Design review of the part built by this model. Coordinates are the model's own, in mm. A direction names the side the tool comes from. Coordinates: 2 decimals unless noted, no trailing zeros. Loops run counter-clockwise (first coordinate to the right, second up) from the corner with the lowest first, then second, coordinate; pieces in that order, holes last. Notation, with made-up numbers: (-40, -20) -> (-21, -20) arc R34 cw to (-21, 12) -> close; hole circle Ø2 at (-30, 62). An arc over 180 degrees is marked (long way). Use CSV: the item, a comma, the result in double quotes.
```python
from build123d import *

# Parameters (mm, degrees)
SKETCH1_W                                = 34
SKETCH1_H                                = 45
BASE_EXTRUDE_DEPTH                       = 16
CUT_EXTRUDE1_DEPTH                       = 56.951622292
CBORE_FOR_M5_HEX_HEAD_SCREW1_D           = 6.6
CBORE_FOR_M5_HEX_HEAD_SCREW1_CBORE_D     = 12
CBORE_FOR_M5_HEX_HEAD_SCREW1_CBORE_DEPTH = 6
SKETCH3_R                                = 3
CUT_EXTRUDE4_DEPTH                       = 25
CHAMFER3_SIZE                            = 2
CHAMFER4_SIZE                            = 2
CBORE_FOR_M5_HEX_HEAD_SCREW2_D           = 6.6
CBORE_FOR_M5_HEX_HEAD_SCREW2_CBORE_D     = 12
CBORE_FOR_M5_HEX_HEAD_SCREW2_CBORE_DEPTH = 6
FILLET1_R                                = 1
FILLET2_R                                = 1
SKETCH13_W                               = 37.795873191
SKETCH13_H                               = 5.669380978
CUT_EXTRUDE5_DEPTH                       = 56.951622292


with BuildPart() as part:
    # Sketch1 → Base-Extrude (new body)
    with BuildSketch(Plane.XY):
        with Locations((0, 28.348638498)):
            Rectangle(SKETCH1_W, SKETCH1_H)
    extrude(amount=BASE_EXTRUDE_DEPTH)

    # Sketch2 → Cut-Extrude1 (cut, through all)
    with BuildSketch(Plane.XY.offset(16)):
        Polygon((-4, 38.848638498), (4, 38.848638498), (4, 42.848638498), (12, 50.848638498), (-12, 50.848638498), (-4, 42.848638498), align=None)
    extrude(amount=-CUT_EXTRUDE1_DEPTH, mode=Mode.SUBTRACT)

    # CBORE for M5 Hex Head Screw1 (through all)
    with Locations(Plane.XY.offset(16)):
        with Locations((7.5, 30.848638498)):
            CounterBoreHole(CBORE_FOR_M5_HEX_HEAD_SCREW1_D / 2, CBORE_FOR_M5_HEX_HEAD_SCREW1_CBORE_D / 2, CBORE_FOR_M5_HEX_HEAD_SCREW1_CBORE_DEPTH)

    # Sketch3 → Cut-Extrude4 (cut)
    with BuildSketch(Plane.XY.offset(16)):
        with Locations((-7.5, 30.848638498)):
            Circle(SKETCH3_R)
        with Locations((7.5, 15.848638498)):
            Circle(SKETCH3_R)
    extrude(amount=-CUT_EXTRUDE4_DEPTH, mode=Mode.SUBTRACT)

    # Chamfer3
    chamfer3_edges = [part.edges().sort_by_distance(p)[0] for p in [
        (-10.5, 30.848638498, 16),
        (4.5, 15.848638498, 16),
    ]]
    chamfer(chamfer3_edges, length=CHAMFER3_SIZE)

    # Chamfer4
    chamfer4_edges = [part.edges().sort_by_distance(p)[0] for p in [
        (-10.5, 30.848638498, 0),
        (4.5, 15.848638498, 0),
    ]]
    chamfer(chamfer4_edges, length=CHAMFER4_SIZE)

    # CBORE for M5 Hex Head Screw2 (through all)
    with Locations(Plane.XY.offset(16)):
        with Locations((-7.5, 15.848638498)):
            CounterBoreHole(CBORE_FOR_M5_HEX_HEAD_SCREW2_D / 2, CBORE_FOR_M5_HEX_HEAD_SCREW2_CBORE_D / 2, CBORE_FOR_M5_HEX_HEAD_SCREW2_CBORE_DEPTH)

    # Fillet1
    fillet1_edges = [part.edges().sort_by_distance(p)[0] for p in [
        (-4, 38.848638498, 8),
    ]]
    fillet(fillet1_edges, radius=FILLET1_R)

    # Fillet2
    fillet2_edges = [part.edges().sort_by_distance(p)[0] for p in [
        (4, 38.848638498, 8),
    ]]
    fillet(fillet2_edges, radius=FILLET2_R)

    # Sketch13 → Cut-Extrude5 (cut, through all)
    with BuildSketch(Plane.XY.offset(16)):
        with Locations((-0.227198085, 51.199908502)):
            Rectangle(SKETCH13_W, SKETCH13_H)
    extrude(amount=-CUT_EXTRUDE5_DEPTH, mode=Mode.SUBTRACT)


solid = part.part
```
Item 1: Draft analysis for pull direction Y (two halves, no side actions). For faces 1 (the face through (7.93, 34.12, 4.93)), 2 (the face through (0, 27, 16)), 3 (the face through (-13, 48.365, 8)), 4 (the face through (0, 5.849, 8)), state which applies: pulls with the +Y half, pulls with the -Y half, needs draft (parallel to the pull), parting line crosses it, or undercut.
Checked values:
face 1,"undercut"
face 2,"needs draft"
face 3,"pulls with the +Y half"
face 4,"pulls with the -Y half"
Item 2: Add section D-D (y = 29.5). State how many separate pieces and enclosed holes the cut face has, then the cut area to 3 significant figures.
Checked values:
separate pieces,"3"
enclosed holes,"0"
area,"319 mm^2"
Item 3: To check wall thickness, follow line 1 along Y through (x, z) = (7.5, 12); line 2 along X through (y, z) = (42, 1.25); line 3 along Y through (x, z) = (6.5, 2.5). State the ranges of each line that lie inside material, in increasing order.
Checked values:
line 1,"5.85 to 12.85, 18.85 to 24.85, 36.85 to 46.35"
line 2,"-17 to -4, 4 to 17"
line 3,"5.85 to 13.02, 18.68 to 27.7, 33.99 to 45.35"
Item 4: Clearance check with flat-ended pins moving along their axes: pin 1 (10.5 mm diameter, centred on x = 7.5, y = 30.85, fed in from +Z); pin 2 (6 mm diameter, centred on x = 4.5, z = 9.5, fed in from +Y); pin 3 (6.5 mm diameter, centred on x = -1, z = 5.5, fed in from +Y). State where each tip first meets the part, or that it passes through.
Checked values:
pin 1,"z = 10"
pin 2,"y = 46.35"
pin 3,"y = 43.1"
Item 5: Add section A-A (x = 7.5). Give the boundary of the cut face in (y, z), then the cut area to 3 significant figures.
Checked values:
outline,"(5.85, 0) -> (10.85, 0) -> (12.85, 2) -> (12.85, 14) -> (10.85, 16) -> (5.85, 16) -> close; (18.85, 2) -> (20.85, 0) -> (27.55, 0) -> (27.55, 10) -> (24.85, 10) -> (24.85, 16) -> (20.85, 16) -> (18.85, 14) -> close; (34.15, 0) -> (46.35, 0) -> (46.35, 16) -> (36.85, 16) -> (36.85, 10) -> (34.15, 10) -> close"
area,"406 mm^2"
Item 6: Add section C-C (x = -2). Give the boundary of the cut face in (y, z).
Checked values:
outline,"(5.85, 0) -> (38.85, 0) -> (38.85, 16) -> (18.25, 16) -> (18.25, 10) -> (13.45, 10) -> (13.45, 16) -> (5.85, 16) -> close"
Item 7: Add section B-B (z = 10.5). Give the boundary of the cut face in (x, y).
Checked values:
outline,"(-17, 5.85) -> (17, 5.85) -> (17, 48.37) -> (9.52, 48.37) -> (4, 42.85) -> (4, 39.85) arc R1 cw to (3, 38.85) -> (-3, 38.85) arc R1 cw to (-4, 39.85) -> (-4, 42.85) -> (-9.52, 48.37) -> (-17, 48.37) -> close; hole circle Ø12 at (-7.5, 15.85); hole circle Ø6 at (-7.5, 30.85); hole circle Ø12 at (7.5, 30.85); hole circle Ø6 at (7.5, 15.85)"
Item 8: Machinability: for faces 5 (the face through (6.719, 36.798, 13.042)), 6 (the face through (-7.91, 33.95, 1.87)), 7 (the face through (0, 38.849, 8)), which of the approach directions +Z, -Z, +X, -X, +Y, -Y give a long, thin tool a straight path to every point of the face, cutting with its end or side? Answer none if there is none.
Checked values:
face 5,"+Z"
face 6,"-Z"
face 7,"+Z, -Z, +Y"
